Check sheet for the modelled part. Datum: model origin and axes. Units: mm. A direction names the side the tool comes from. Round coordinates to 2 decimals unless told otherwise and drop trailing zeros. Loops run counter-clockwise (first coordinate to the right, second up) from the corner with the lowest first, then second, coordinate; pieces in that order, holes last. Notation, with made-up numbers: (48.5, 55.25) - (61.5, 55.25) arc R23 cw to (61.5, 90.25) - close; hole circle Ø3 at (16.25, -33.5). An arc over 180 degrees is marked (long way). Answer in a Markdown table with one row per item. Add a question column.
(1) Thickness scan on line 1 along X through (y, z) = (239, 0); line 2 along Z through (x, y) = (-21.5, 341); line 3 along X through (y, z) = (-79.5, -40). Record the ranges inside material, lowest first.
(2) Gauge pin test, flat ends, axial feed: pin 1 (6 mm diameter, centred on x = -42.5, z = 57.5, fed in from -Y); pin 2 (4 mm diameter, centred on y = -48, z = 53, fed in from -X); pin 3 (10 mm diameter, centred on x = 12, y = 179, fed in from -Z). Record the tip position at first contact, or that the pin passes through.
(3) Mould release check, pull along X, two halves, no side actions. Record for faces 1 (the flat face through (63, 370.012, 17)), 2 (the cylindrical face through (68.756, 113.834, 35.762)), 3 (the cylindrical face through (56.133, 122.904, -12.465)): +X half, -X half, draft (parallel to the pull), parting line (faces both ways), or undercut.
(4) Cross-section at C-C on y = -56. Enter the section's corners in (x, z).
(5) Cross-section at B-B on x = 0. Enter the section's corners in (y, z).
(6) Access from +Z, -Z, +X, -X, +Y, -Y to the whole of each face (thin tool, end or side, straight path). Record for faces 4 (the flat face through (63, -149.618, 18)), 5 (the cylindrical face through (-19.52, 420.71, 62)), 6 (the flat face through (57.5, 470.012, 4.5)).
(7) Cross-section at A-A on z = 0. Enter the section's corners in (x, y).
from build123d import *


with BuildPart() as part:
    # 草图1 → 旋转1 (revolve)
    with BuildSketch(Plane.XY, mode=Mode.PRIVATE) as revolve_1_sk:
        Polygon((57.5, 470.011904762), (57.5, -214.618095238), (65, -214.618095238), (65, -149.618095238), (77.5, -149.618095238), (77.5, 370.011904762), (65, 370.011904762), (65, 470.011904762), align=None)
    revolve(revolve_1_sk.sketch.rotate(Axis((0, 125.678571429, 0), (0, -1, 0)), 90), axis=Axis((0, 125.678571429, 0), (0, -1, 0)))


solid = part.part
Answers:
| question | item | result |
|---|---|---|
| 1 | line 1 | x = -77.5 to -57.5, 57.5 to 77.5 |
| 1 | line 2 | z = -74.46 to -53.33, 53.33 to 74.46 |
| 1 | line 3 | x = -66.38 to -41.31, 41.31 to 66.38 |
| 2 | pin 1 | stops at y = -149.62 |
| 2 | pin 2 | stops at x = -58.35 |
| 2 | pin 3 | stops at z = -77.18 |
| 3 | face 1 | draft |
| 3 | face 2 | parting line |
| 3 | face 3 | undercut |
| 4 | outline | circle Ø155 at (0, 0); hole circle Ø115 at (0, 0) |
| 5 | outline | (-214.62, -65) - (-149.62, -65) - (-149.62, -77.5) - (370.01, -77.5) - (370.01, -65) - (470.01, -65) - (470.01, -57.5) - (-214.62, -57.5) - close; (-214.62, 57.5) - (470.01, 57.5) - (470.01, 65) - (370.01, 65) - (370.01, 77.5) - (-149.62, 77.5) - (-149.62, 65) - (-214.62, 65) - close |
| 6 | face 4 | -Y |
| 6 | face 5 | +Y |
| 6 | face 6 | +Z, -Z, +X, -X, +Y |
| 7 | outline | (-77.5, -149.62) - (-65, -149.62) - (-65, -214.62) - (-57.5, -214.62) - (-57.5, 470.01) - (-65, 470.01) - (-65, 370.01) - (-77.5, 370.01) - close; (57.5, -214.62) - (65, -214.62) - (65, -149.62) - (77.5, -149.62) - (77.5, 370.01) - (65, 370.01) - (65, 470.01) - (57.5, 470.01) - close |
